Geometry check sheet. Reference: the model listing, model coordinates, mm. Face numbers are marked on the shaded views. Round coordinates to 2 decimals unless told otherwise and drop trailing zeros. Order: outer loops, then holes, each group sorted by start corner. A loop starts at its lowest first (then second) coordinate and runs counter-clockwise, first axis right, second up. Notation, with made-up numbers: (39.5, -8.5) - (58.5, -8.5) arc R25 cw to (58.5, 19.5) - close; hole circle Ø11 at (-23.5, 23.5). An arc over 180 degrees is marked (long way). One line per question, with ' | ' between items. Start each with the question number.
Q1. Sectioned sample at A-A, the plane y = 0. Enter the section's corners in (x, z).
Q2. Sectioned sample at D-D, the plane y = 3.5. Enter the section's corners in (x, z), then the cut area to 3 significant figures.
Q3. Sectioned sample at C-C, the plane x = 25. Enter the section's corners in (y, z).
Q4. Gauge pin test, flat ends, axial feed: P1, Ø1, axis at x = -21.5, y = -2.5, coming from the +Z side; P2, Ø1.5, axis at y = -1, z = 3, coming from the +X side; P3, Ø3, axis at y = -2.5, z = 2, coming from the -X side. Record the tip position at first contact, or that the pin passes through.
Q5. Mould release check, pull along Y, two halves, no side actions. Record for the marked faces 1, 2 and 3: +Y half, -Y half, draft (parallel to the pull), parting line (faces both ways), or undercut.
Q6. Material ranges on line 1 along Y through (x, z) = (-23.5, 4.45); line 2 along X through (y, z) = (2.75, 5.65); line 3 along X through (y, z) = (-2, 3.05), recorded low to high.
Q7. Sectioned sample at B-B, the plane z = 5.35. Enter the section's corners in (x, y).
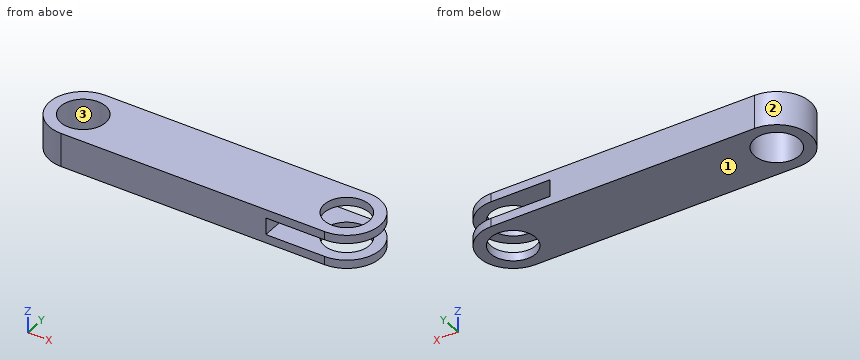
```python
from build123d import *

# Parameters (mm, degrees)
BOSS_EXTRUDE1_DEPTH = 6
SKETCH2_W           = 33
SKETCH2_H           = 3
CUT_EXTRUDE1_DEPTH  = 35
SKETCH3_R           = 4
CUT_EXTRUDE2_DEPTH  = 35


with BuildPart() as part:
    # Sketch1 → Boss-Extrude1 (new body)
    with BuildSketch(Plane.XY):
        with BuildLine():
            Line((23.5, -6), (-23.5, -6))
            ThreePointArc((-23.5, -6), (-29.5, 0), (-23.5, 6))
            Line((-23.5, 6), (23.5, 6))
            ThreePointArc((23.5, 6), (29.5, 0), (23.5, -6))
        make_face()
    extrude(amount=BOSS_EXTRUDE1_DEPTH)

    # Sketch2 → Cut-Extrude1 (cut)
    with BuildSketch(Plane(origin=(0, 6, 0), x_dir=(1, 0, 0), z_dir=(0, 1, 0))):
        with Locations((29.5, -3)):
            Rectangle(SKETCH2_W, SKETCH2_H)
    extrude(amount=-CUT_EXTRUDE1_DEPTH, mode=Mode.SUBTRACT)

    # Sketch3 → Cut-Extrude2 (cut)
    with BuildSketch(Plane.XY.offset(6)):
        with Locations((23.5, 0)):
            Circle(SKETCH3_R)
        with Locations((-23.5, 0)):
            Circle(SKETCH3_R)
    extrude(amount=-CUT_EXTRUDE2_DEPTH, mode=Mode.SUBTRACT)


solid = part.part
```
Determined:
1) outline: (-29.5, 0) - (-27.5, 0) - (-27.5, 6) - (-29.5, 6) - close; (-19.5, 0) - (19.5, 0) - (19.5, 1.5) - (13, 1.5) - (13, 4.5) - (19.5, 4.5) - (19.5, 6) - (-19.5, 6) - close; (27.5, 0) - (29.5, 0) - (29.5, 1.5) - (27.5, 1.5) - close; (27.5, 4.5) - (29.5, 4.5) - (29.5, 6) - (27.5, 6) - close
2) outline: (-28.37, 0) - (-25.44, 0) - (-25.44, 6) - (-28.37, 6) - close; (-21.56, 0) - (21.56, 0) - (21.56, 1.5) - (13, 1.5) - (13, 4.5) - (21.56, 4.5) - (21.56, 6) - (-21.56, 6) - close; (25.44, 0) - (28.37, 0) - (28.37, 1.5) - (25.44, 1.5) - close; (25.44, 4.5) - (28.37, 4.5) - (28.37, 6) - (25.44, 6) - close | area: 260 mm2
3) outline: (-5.81, 0) - (-3.71, 0) - (-3.71, 1.5) - (-5.81, 1.5) - close; (-5.81, 4.5) - (-3.71, 4.5) - (-3.71, 6) - (-5.81, 6) - close; (3.71, 0) - (5.81, 0) - (5.81, 1.5) - (3.71, 1.5) - close; (3.71, 4.5) - (5.81, 4.5) - (5.81, 6) - (3.71, 6) - close
4) P1: passes through | P2: stops at x = 13 | P3: stops at x = -29.42
5) face 1: draft | face 2: parting line | face 3: undercut
6) line 1: y = -6 to -4, 4 to 6 | line 2: x = -28.83 to -26.4, -20.6 to 20.6, 26.4 to 28.83 | line 3: x = -29.16 to -26.96, -20.04 to 13
7) outline: (-23.5, -6) - (23.5, -6) arc R6 ccw to (23.5, 6) - (-23.5, 6) arc R6 ccw to start; hole circle Ø8 at (-23.5, 0); hole circle Ø8 at (23.5, 0)
